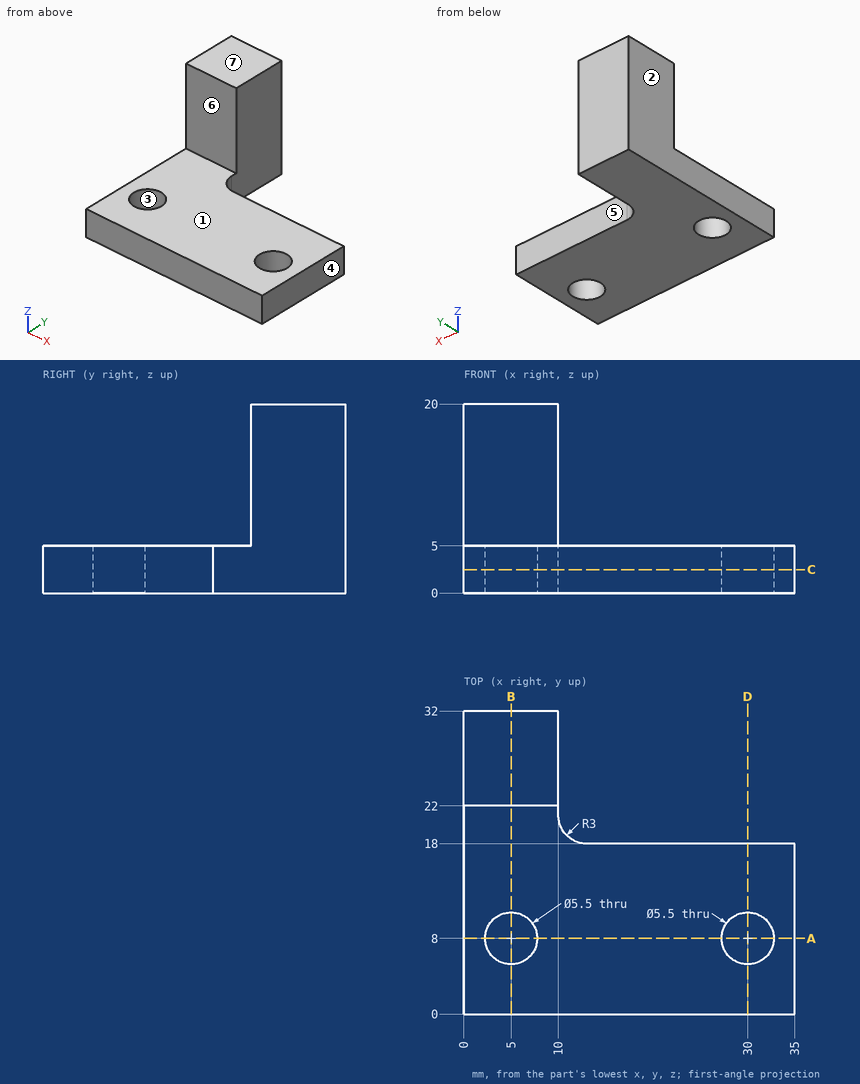
Job drawing, mm, ordinate dimensions from the low corner. One solid piece. A direction names the side the tool comes from. Give positions to 0.01 mm unless a question says otherwise; leave off trailing zeros. Order: outer loops, then holes, each group sorted by start corner. A loop starts at its lowest first (then second) coordinate and runs counter-clockwise, first axis right, second up. Notation, with made-up numbers: (30, 32.5) - (57, 32.5) arc R17 cw to (57, 48.5) - close; hole circle Ø3 at (49, -38.5). An arc over 180 degrees is marked (long way). One line per question, with ' | ' between items.
1. Which spindle directions (+Z, -Z, +X, -X, +Y, -Y) get a long thin tool onto all of the face, cutting with end or side? Do the marked faces 5, 6 and 7. Say none if no direction does.
Filled in:
face 5: +Z, -Z, +X, +Y | face 6: +Z, +X, -X, -Y | face 7: +Z, +X, -X, +Y, -Y
2. Band-saw the part on A-A on y = 8. List the corners of the cut face in (x, z).
Filled in:
outline: (0, 0) - (2.25, 0) - (2.25, 5) - (0, 5) - close; (7.75, 0) - (27.25, 0) - (27.25, 5) - (7.75, 5) - close; (32.75, 0) - (35, 0) - (35, 5) - (32.75, 5) - close
3. Drill centre lines: probe 1 along Y at (x, z) = (30, 2.5); probe 2 along Y at (x, z) = (9.5, 12); probe 3 along Z at (x, y) = (13, 12.5). Where is each one in solid material? Low to high.
Filled in:
probe 1: 0 to 5.25, 10.75 to 18 | probe 2: 22 to 32 | probe 3: 0 to 5
4. Band-saw the part on D-D on x = 30. List the corners of the cut face in (y, z).
Filled in:
outline: (0, 0) - (5.25, 0) - (5.25, 5) - (0, 5) - close; (10.75, 0) - (18, 0) - (18, 5) - (10.75, 5) - close
5. Drop flat-ended pins along their axis: P1, Ø2.5, axis at x = 23.5, z = 2, coming from the +Y side; P2, Ø8, axis at y = 23.5, z = 2.5, coming from the +X side; P3, Ø5.5, axis at y = 24, z = 9, coming from the +X side. Give the stop position or say it passes through.
Filled in:
P1: y = 18 | P2: x = 10.4 | P3: x = 10
6. Band-saw the part on C-C on z = 2.5. List the corners of the cut face in (x, y), then the cut area to 3 significant figures.
Filled in:
outline: (0, 0) - (35, 0) - (35, 18) - (13, 18) arc R3 cw to (10, 21) - (10, 32) - (0, 32) - close; hole circle Ø5.5 at (5, 8); hole circle Ø5.5 at (30, 8) | area: 724 mm²
7. Band-saw the part on B-B on x = 5. List the corners of the cut face in (y, z), then the cut area to 4 significant figures.
Filled in:
outline: (0, 0) - (5.25, 0) - (5.25, 5) - (0, 5) - close; (10.75, 0) - (32, 0) - (32, 20) - (22, 20) - (22, 5) - (10.75, 5) - close | area: 282.5 mm²
8. Pull direction X, two halves, no side cores. Call the marked faces 1, 2, 3 and 4: +X half, -X half, draft (parallel to the pull), parting line (faces both ways), or undercut.
Filled in:
face 1: draft | face 2: -X half | face 3: undercut | face 4: +X half
